For this review, take the finished solid that the model builds, in its own axes (mm). A direction names the side the tool comes from. Round coordinates to 2 decimals unless told otherwise and drop trailing zeros. Write each loop counter-clockwise with the first axis right and the second up, starting at its lowest first coordinate (ties: lowest second). Pieces come first, ordered by that corner, then holes. Notation, with made-up numbers: M 27,33 L 78,33 A21 cw 78,63 Z; hole C -4.75,-35.5 d10. An arc over 180 degrees is marked long. Use one line per item in the form item = value. Start each with the question number.
Item 1: Add section D-D (x = 10.5). State the section outline as (y, z) points, and give its area (3 significant figures).
Item 2: Add section B-B (y = 0). State the section outline as (x, z) points.
Item 3: For faces 1 (the flat face through (0, -5, 2)), 2 (the flat face through (6.5, -3, 2)), 3 (the flat face through (-4, 0, 0)), list the 3-axis set-ups (+Z, -Z, +X, -X, +Y, -Y) from which the entire face can be reached by the end or side of a thin tool; tool diameter is ignored.
Item 4: Add section C-C (x = -0.5). State the section outline as (y, z) points, and give its area (3 significant figures).
Item 5: Add section A-A (z = 0). State the section outline as (x, y) points, and give its area (3 significant figures).
Item 6: For line 1 (X direction, y = 2.75, z = -3); line 2 (Z direction, x = 3.25, y = 3); line 3 (Y direction, x = 14.25, z = -2), list the stretches that pass through material, from the lowest coordinate up. Write a range as [from, to].
Item 7: For P1, Ø1, axis at x = -5, z = 1.5, coming from the +Y side; P2, Ø1.5, axis at x = 5.5, y = -2, coming from the -Z side; P3, Ø6, axis at x = 4, y = -2, coming from the +Z side, all flat-tipped, find the tip position at first contact; note any pin that passes through.
Item 8: Draft analysis for pull direction Y (two halves, no side actions). For faces 4 (the flat face through (-5, 0.6, 0)), 5 (the cylindrical face through (2.22, -4.88, 1.08)), 6 (the flat face through (-6, 3, 0)), 7 (the flat face through (-5, -0.6, 0)), state which applies: released by +Y, released by -Y, zero draft, split by the parting line, or undercut.
from build123d import *

# Parameters (mm, degrees)
SKETCH_2_R          = 5
EXTRUDE_1_DEPTH     = 5
SKETCH_5_R          = 6.5
EXTRUDE_2_DEPTH     = 6
SKETCH_6_W          = 30
SKETCH_6_H          = 1.2
CUT_EXTRUDE_1_DEPTH = 2
SKETCH_7_R          = 4
EXTRUDE_3_DEPTH     = 15
CHAMFER_3_SIZE      = 0.5
SKETCH_8_W          = 1.5
SKETCH_8_H          = 1.794916968


with BuildPart() as part:
    # 草图2 → 凸台-拉伸1 (new body)
    with BuildSketch(Plane(origin=(0, 0, 0), x_dir=(0, 0, -1), z_dir=(1, 0, 0))):
        Circle(SKETCH_2_R)
    extrude(amount=EXTRUDE_1_DEPTH)

    # 草图5 → 凸台-拉伸2 (add)
    with BuildSketch(Plane.ZY):
        Circle(SKETCH_5_R)
    extrude(amount=EXTRUDE_2_DEPTH)

    # 草图6 → 切除-拉伸1 (cut)
    with BuildSketch(Plane.ZY.offset(6)):
        Rectangle(SKETCH_6_W, SKETCH_6_H)
    extrude(amount=-CUT_EXTRUDE_1_DEPTH, mode=Mode.SUBTRACT)

    # 草图7 → 凸台-拉伸3 (add)
    with BuildSketch(Plane(origin=(5, 0, 0), x_dir=(0, 0, -1), z_dir=(1, 0, 0))):
        Circle(SKETCH_7_R)
    extrude(amount=EXTRUDE_3_DEPTH)

    # 倒角3
    chamfer_3_edges = [part.edges().sort_by_distance(p)[0] for p in [
        (20, 0, 4),
        (5, 0, 5),
    ]]
    chamfer(chamfer_3_edges, length=CHAMFER_3_SIZE)

    # 草图8 → 切除-旋转1 (revolve, cut)
    with BuildSketch(Plane(origin=(0, 0, 0), x_dir=(1, 0, 0), z_dir=(0, 1, 0)), mode=Mode.PRIVATE) as cut_revolve_1_sk:
        with Locations((5.75, 4.147458484)):
            Rectangle(SKETCH_8_W, SKETCH_8_H)
    revolve(cut_revolve_1_sk.sketch.rotate(Axis((0, 0, 0), (1, 0, 0)), 180), axis=Axis((0, 0, 0), (1, 0, 0)), mode=Mode.SUBTRACT)


solid = part.part
Calculated:
q1.outline = C 0,0 d8
q1.area = 50.3 mm^2
q2.outline = M -4,-6.5 L 0,-6.5 L 0,-5 L 4.5,-5 L 5,-4.5 L 5,-3.25 L 6.5,-3.25 L 6.5,-4 L 19.5,-4 L 20,-3.5 L 20,3.5 L 19.5,4 L 6.5,4 L 6.5,3.25 L 5,3.25 L 5,4.5 L 4.5,5 L 0,5 L 0,6.5 L -4,6.5 Z
q3.face_1 = +X
q3.face_2 = none
q3.face_3 = +Z, -Z, -X
q4.outline = C 0,0 d13
q4.area = 133 mm^2
q5.outline = M -6,-6.5 L 0,-6.5 L 0,-5 L 4.5,-5 L 5,-4.5 L 5,-3.25 L 6.5,-3.25 L 6.5,-4 L 19.5,-4 L 20,-3.5 L 20,3.5 L 19.5,4 L 6.5,4 L 6.5,3.25 L 5,3.25 L 5,4.5 L 4.5,5 L 0,5 L 0,6.5 L -6,6.5 L -6,0.6 L -4,0.6 L -4,-0.6 L -6,-0.6 Z
q5.area = 243 mm^2
q6.line_1 = [-6, 5]
q6.line_2 = [-4, 4]
q6.line_3 = [-3.46, 3.46]
q7.P1 = 6.42
q7.P2 = -4.37
q7.P3 = 5
q8.face_4 = undercut
q8.face_5 = split by the parting line
q8.face_6 = zero draft
q8.face_7 = undercut
